Build history of the part. All positions in model axes, mm. Face numbers are marked on the shaded views. A direction names the side the tool comes from. Give positions to 0.01 mm unless a question says otherwise; leave off trailing zeros. Order: outer loops, then holes, each group sorted by start corner. A loop starts at its lowest first (then second) coordinate and runs counter-clockwise, first axis right, second up. Notation, with made-up numbers: (-14.75, 69.25) -> (-7.75, 69.25) arc R32 cw to (-7.75, 105.25) -> close; hole circle Ø7 at (-13, 28). An arc over 180 degrees is marked (long way). Use a Markdown table: item, result. Add a question column.
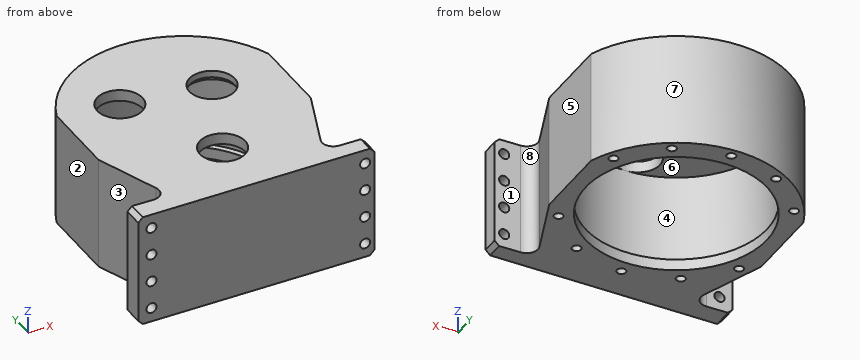
```python
from build123d import *

# Parameters (mm, degrees)
SKETCH1_R           = 50
BOSS_EXTRUDE1_DEPTH = 50
SKETCH2_R           = 42.5
CUT_EXTRUDE1_DEPTH  = 45
SKETCH3_R           = 12.5
CUT_EXTRUDE2_DEPTH  = 2
SKETCH4_R           = 10
CUT_EXTRUDE3_DEPTH  = 84.815273071
BOSS_EXTRUDE2_DEPTH = 50
CUT_EXTRUDE4_DEPTH  = 96.077733998
SKETCH7_R           = 2.25
CUT_EXTRUDE5_DEPTH  = 20
FILLET1_R           = 5
FILLET2_R           = 5
CHAMFER1_SIZE       = 2
SKETCH8_R           = 4
CUT_EXTRUDE6_DEPTH  = 1
SKETCH9_R           = 11.5
CUT_EXTRUDE8_DEPTH  = 2
SKETCH10_R          = 42.5
SKETCH10_R_2        = 40
BOSS_EXTRUDE3_DEPTH = 5
SKETCH11_R          = 2
CUT_EXTRUDE9_DEPTH  = 8


with BuildPart() as part:
    # Sketch1 → Boss-Extrude1 (new body)
    with BuildSketch(Plane.XY):
        Circle(SKETCH1_R)
    extrude(amount=BOSS_EXTRUDE1_DEPTH)

    # Sketch2 → Cut-Extrude1 (cut)
    with BuildSketch(Plane(origin=(0, 0, 0), x_dir=(-1, 0, 0), z_dir=(0, 0, -1))):
        Circle(SKETCH2_R)
    extrude(amount=-CUT_EXTRUDE1_DEPTH, mode=Mode.SUBTRACT)

    # Sketch3 → Cut-Extrude2 (cut)
    with BuildSketch(Plane(origin=(0, 0, 45), x_dir=(-1, 0, 0), z_dir=(0, 0, -1))):
        Circle(SKETCH3_R)
    extrude(amount=-CUT_EXTRUDE2_DEPTH, mode=Mode.SUBTRACT)

    # Sketch4 → Cut-Extrude3 (cut, through all)
    with BuildSketch(Plane(origin=(0, 0, 45), x_dir=(-1, 0, 0), z_dir=(0, 0, -1))):
        with Locations((-17, 8.485281374)):
            Circle(SKETCH4_R)
        with Locations((21.2, 13.24990566)):
            Circle(SKETCH4_R)
        with Locations((0, -32.5)):
            Circle(SKETCH4_R)
    extrude(amount=-CUT_EXTRUDE3_DEPTH, mode=Mode.SUBTRACT)

    # Sketch5 → Boss-Extrude2 (add)
    with BuildSketch(Plane(origin=(0, 0, 0), x_dir=(-1, 0, 0), z_dir=(0, 0, -1))):
        with BuildLine():
            Line((-46.833609462, -17.510369063), (-33.74764568, -52.510369063))
            Line((-33.74764568, -52.510369063), (-52.5, -52.510369063))
            Line((-52.5, -52.510369063), (-52.5, -59.989582371))
            Line((-52.5, -59.989582371), (52.5, -61.510369063))
            Line((52.5, -61.510369063), (52.5, -52.510369063))
            Line((52.5, -52.510369063), (33.74764568, -52.510369063))
            Line((33.74764568, -52.510369063), (46.833609462, -17.510369063))
            ThreePointArc((46.833609462, -17.510369063), (0, -50), (-46.833609462, -17.510369063))
        make_face()
    extrude(amount=-BOSS_EXTRUDE2_DEPTH)

    # Sketch6 → Cut-Extrude4 (cut, through all)
    with BuildSketch(Plane(origin=(0, 0, 0), x_dir=(-1, 0, 0), z_dir=(0, 0, -1))):
        with BuildLine():
            Line((-46.833609462, -17.510369063), (-46.833609462, 17.510369063))
            ThreePointArc((-46.833609462, 17.510369063), (-50, 0), (-46.833609462, -17.510369063))
        make_face()
        with BuildLine():
            Line((46.833609462, -17.510369063), (46.833609462, 17.510369063))
            ThreePointArc((46.833609462, 17.510369063), (50, 0), (46.833609462, -17.510369063))
        make_face()
    extrude(amount=-CUT_EXTRUDE4_DEPTH, mode=Mode.SUBTRACT)

    # Sketch7 → Cut-Extrude5 (cut)
    with BuildSketch(Plane(origin=(0.879698836, -60.737234438, 0), x_dir=(0.9998951279661363, 0.014482163843290402, 0), z_dir=(0.014482163843290404, -0.9998951279661364, 0))):
        with Locations((-47.5, 43.75)):
            Circle(SKETCH7_R)
        with Locations((-47.5, 31.25)):
            Circle(SKETCH7_R)
        with Locations((47.5, 31.25)):
            Circle(SKETCH7_R)
        with Locations((47.5, 43.75)):
            Circle(SKETCH7_R)
        with Locations((47.5, 18.75)):
            Circle(SKETCH7_R)
        with Locations((47.5, 6.25)):
            Circle(SKETCH7_R)
        with Locations((-47.5, 18.75)):
            Circle(SKETCH7_R)
        with Locations((-47.5, 6.25)):
            Circle(SKETCH7_R)
    extrude(amount=-CUT_EXTRUDE5_DEPTH, mode=Mode.SUBTRACT)

    # Fillet1
    fillet1_edges = [part.edges().sort_by_distance(p)[0] for p in [
        (33.74764568, -52.510369063, 25),
    ]]
    fillet(fillet1_edges, radius=FILLET1_R)

    # Fillet2
    fillet2_edges = [part.edges().sort_by_distance(p)[0] for p in [
        (-33.74764568, -52.510369063, 25),
    ]]
    fillet(fillet2_edges, radius=FILLET2_R)

    # Chamfer1
    chamfer1_edges = [part.edges().sort_by_distance(p)[0] for p in [
        (-52.5, -57.010369063, 50),
        (52.5, -56.249975717, 50),
        (52.5, -56.249975717, 0),
        (-52.5, -57.010369063, 0),
    ]]
    chamfer(chamfer1_edges, length=CHAMFER1_SIZE)

    # Sketch8 → Cut-Extrude6 (cut)
    with BuildSketch(Plane(origin=(0, 0, 47), x_dir=(-1, 0, 0), z_dir=(0, 0, -1))):
        Circle(SKETCH8_R)
    extrude(amount=-CUT_EXTRUDE6_DEPTH, mode=Mode.SUBTRACT)

    # Sketch9 → Cut-Extrude8 (cut)
    with BuildSketch(Plane(origin=(0, 0, 45), x_dir=(-1, 0, 0), z_dir=(0, 0, -1))):
        with Locations((-17, 8.485281374)):
            Circle(SKETCH9_R)
    extrude(amount=-CUT_EXTRUDE8_DEPTH, mode=Mode.SUBTRACT)

    # Sketch10 → Boss-Extrude3 (add)
    with BuildSketch(Plane(origin=(0, 0, 0), x_dir=(-1, 0, 0), z_dir=(0, 0, -1))):
        Circle(SKETCH10_R)
        Circle(SKETCH10_R_2, mode=Mode.SUBTRACT)
    extrude(amount=-BOSS_EXTRUDE3_DEPTH)

    # Sketch11 → Cut-Extrude9 (cut)
    with BuildSketch(Plane(origin=(0, 0, 0), x_dir=(-1, 0, 0), z_dir=(0, 0, -1))):
        with Locations((0, 46)):
            Circle(SKETCH11_R)
        with Locations((23, 39.837168574)):
            Circle(SKETCH11_R)
        with Locations((39.837168574, 23)):
            Circle(SKETCH11_R)
        with Locations((-23, 39.837168574)):
            Circle(SKETCH11_R)
        with Locations((-39.837168574, 23)):
            Circle(SKETCH11_R)
        with Locations(Location((39.837168574, -23, 0), (0, 0, 180))):
            Circle(SKETCH11_R)
        with Locations(Location((23, -39.837168574, 0), (0, 0, 180))):
            Circle(SKETCH11_R)
        with Locations(Location((0, -46, 0), (0, 0, 180))):
            Circle(SKETCH11_R)
        with Locations(Location((-23, -39.837168574, 0), (0, 0, 180))):
            Circle(SKETCH11_R)
        with Locations(Location((-39.837168574, -23, 0), (0, 0, 180))):
            Circle(SKETCH11_R)
    extrude(amount=-CUT_EXTRUDE9_DEPTH, mode=Mode.SUBTRACT)


solid = part.part
```
(1) Band-saw the part on C-C on x = -34.5. Give the cut face in (y, z).
(2) Band-saw the part on D-D on y = -51. Give the cut face in (x, z).
(3) Band-saw the part on B-B on x = 19. Give the cut face in (y, z), plus the area to 3 significant figures.
(4) Band-saw the part on A-A on z = 10. Give the cut face in (x, y).
(5) Pin check, flat tips, straight feed: pin 1 Ø4.5 at (x, y) = (-22.5, 40) entering from -Z; pin 2 Ø18 at (x, y) = (0, -32.5) entering from +Z; pin 3 Ø1.2 at (x, y) = (-40.5, 22) entering from -Z; pin 4 Ø8 at (y, z) = (-14, 21) entering from +X. Stop position of each tip, or through.
(6) Tool access for the marked faces 1, 2, 3, 4 and 5: list every direction of +Z, -Z, +X, -X, +Y, -Y with a clear straight run to the whole face (end or side of a thin tool).
(7) Wall check: probe 1 along Z at (x, y) = (-39, 14); probe 2 along Z at (x, y) = (-11.5, -34); probe 3 along Z at (x, y) = (1, -5.5). Give the ranges that are in metal, low to high.
(8) Mould opens along X. For the marked faces 6, 7 and 8 say: released by +X, released by -X, zero draft, split by the parting line, or undercut.
Response:
| question | item | result |
|---|---|---|
| 1 | outline | (-61.25, 0) -> (-20.24, 0) -> (-20.24, 5) -> (-24.82, 5) -> (-24.82, 45) -> (24.82, 45) -> (24.82, 5) -> (20.24, 5) -> (20.24, 0) -> (36.19, 0) -> (36.19, 50) -> (-61.25, 50) -> close |
| 2 | outline | (-37.37, 0) -> (37.37, 0) -> (37.37, 50) -> (-37.37, 50) -> close |
| 3 | outline | (-60.47, 0) -> (-35.2, 0) -> (-35.2, 5) -> (-38.02, 5) -> (-38.02, 45) -> (-2.84, 45) -> (-2.84, 47) -> (-1.31, 47) -> (-1.31, 50) -> (-60.47, 50) -> close; (18.28, 47) -> (19.81, 47) -> (19.81, 45) -> (38.02, 45) -> (38.02, 5) -> (35.2, 5) -> (35.2, 0) -> (46.25, 0) -> (46.25, 50) -> (18.28, 50) -> close |
| 3 | area | 1,840 mm² |
| 4 | outline | (-52.5, -61.51) -> (52.5, -59.99) -> (52.5, -52.51) -> (40.96, -52.51) arc R5 cw to (36.27, -45.76) -> (46.83, -17.51) -> (46.83, 17.51) arc R50 ccw to (-46.83, 17.51) -> (-46.83, -17.51) -> (-36.27, -45.76) arc R5 cw to (-40.96, -52.51) -> (-52.5, -52.51) -> close; hole circle Ø85 at (0, 0) |
| 5 | pin 1 | stops at z = 0 |
| 5 | pin 2 | stops at z = 5 |
| 5 | pin 3 | stops at z = 8 |
| 5 | pin 4 | stops at x = 46.83 |
| 6 | face 1 | +Z, -Z, +X |
| 6 | face 2 | +Z, -Z, -X, +Y |
| 6 | face 3 | +Z, -Z, -X |
| 6 | face 4 | none |
| 6 | face 5 | +Z, -Z, +X, +Y |
| 7 | probe 1 | z = 0 to 5, 45 to 50 |
| 7 | probe 2 | z = 45 to 50 |
| 7 | probe 3 | z = 47 to 50 |
| 8 | face 6 | undercut |
| 8 | face 7 | split by the parting line |
| 8 | face 8 | released by +X |
